from build123d import *

# Parameters (mm, degrees)
STANCHION_PROFILE_SKETCH_R = 17
STANCHION_BODY_DEPTH       = 33
CORNER_NOTCH_SKETCH_W      = 42
CORNER_NOTCH_SKETCH_H      = 58
CORNER_NOTCH_12X12_DEPTH   = 183.247085025
SLOTTED_BOSS_DEPTH         = 8
HINGE_BARREL_SKETCH_R      = 24
HINGE_BARREL_SKETCH_R_2    = 10
HINGE_BARREL_DEPTH         = 27.5
BARREL_START               = -9
BARREL_GUSSET_DEPTH        = 9
BARREL_RECESS_SKETCH_R     = 17
BARREL_RECESS_CUT_DEPTH    = 6


with BuildPart() as part:
    # Stanchion Profile Sketch → Stanchion Body (new, symmetric)
    with BuildSketch(Plane.XY):
        with BuildLine():
            Line((0, 0), (165, 0))
            Line((165, 0), (165, -12))
            Line((165, -12), (149.032106642, -52.311615965))
            ThreePointArc((149.032106642, -52.311615965), (133.013045842, -68.148401729), (110.513423096, -67.061631974))
            Line((110.513423096, -67.061631974), (0, -12))
            Line((0, -12), (0, 0))
        make_face()
        with Locations((123, -42)):
            Circle(STANCHION_PROFILE_SKETCH_R, mode=Mode.SUBTRACT)
    extrude(amount=STANCHION_BODY_DEPTH, both=True)

    # Corner Notch Sketch → Corner Notch 12x12 (cut, through all)
    with BuildSketch(Plane(origin=(165, 0, 0), x_dir=(0, 0, -1), z_dir=(1, 0, 0))):
        with Locations((0, -41)):
            Rectangle(CORNER_NOTCH_SKETCH_W, CORNER_NOTCH_SKETCH_H)
    extrude(amount=-CORNER_NOTCH_12X12_DEPTH, mode=Mode.SUBTRACT)

    # Slotted Boss Sketch → Slotted Boss (add)
    with BuildSketch(Plane(origin=(0, 0, 0), x_dir=(1, 0, 0), z_dir=(0, 1, 0))):
        with BuildLine():
            Line((105, 16), (141, 16))
            ThreePointArc((141, 16), (157, 0), (141, -16))
            Line((141, -16), (105, -16))
            ThreePointArc((105, -16), (89, 0), (105, 16))
        make_face()
        with BuildLine():
            Line((105, 7.5), (141, 7.5))
            ThreePointArc((141, 7.5), (148.5, 0), (141, -7.5))
            Line((141, -7.5), (105, -7.5))
            ThreePointArc((105, -7.5), (97.5, 0), (105, 7.5))
        make_face(mode=Mode.SUBTRACT)
    extrude(amount=SLOTTED_BOSS_DEPTH)



with BuildPart() as body_2:
    # Hinge Barrel Sketch → Hinge Barrel (new, symmetric)
    with BuildSketch(Plane.XY):
        with Locations((50, 45)):
            Circle(HINGE_BARREL_SKETCH_R)
        with Locations((50, 45)):
            Circle(HINGE_BARREL_SKETCH_R_2, mode=Mode.SUBTRACT)
    extrude(amount=HINGE_BARREL_DEPTH, both=True)


with BuildPart() as part_1:
    add(part.part)

    add(body_2.part)  # Barrel Gusset merges body 2
    # Barrel Gusset Sketch → Barrel Gusset (add)
    with BuildSketch(Plane.XY.offset(27.5).offset(BARREL_START)):
        with BuildLine():
            Line((73.619203331, 49.258313517), (82.5, 0))
            Line((82.5, 0), (16.5, 0))
            Line((16.5, 0), (26.468315489, 49.718031802))
            ThreePointArc((26.468315489, 49.718031802), (49.766012583, 21.001140654), (73.619203331, 49.258313517))
        make_face()
    barrel_gusset = extrude(amount=-BARREL_GUSSET_DEPTH)

    # Barrel Gusset Mirror: Barrel Gusset across plane
    add(barrel_gusset.mirror(Plane.XY))

    # Barrel Recess Sketch → Barrel Recess Cut (cut)
    with BuildSketch(Plane.XY.offset(27.5)):
        with Locations((50, 45)):
            Circle(BARREL_RECESS_SKETCH_R)
    barrel_recess_cut = extrude(amount=-BARREL_RECESS_CUT_DEPTH, mode=Mode.SUBTRACT)

    # Barrel Recess Mirror: Barrel Recess Cut across plane
    add(barrel_recess_cut.mirror(Plane.XY), mode=Mode.SUBTRACT)


solid = part_1.part
Verification items for the finished model (mm, model axes). A direction names the side the tool comes from. Give positions to 0.01 mm unless a question says otherwise; leave off trailing zeros. Order: outer loops, then holes, each group sorted by start corner. A loop starts at its lowest first (then second) coordinate and runs counter-clockwise, first axis right, second up. Notation, with made-up numbers: M 47.5,-20.75 L 67.5,-20.75 A8 ccw 67.5,-10.75 Z; hole C 6,65.5 d1. An arc over 180 degrees is marked long. Answer as a JSON object with one key per item and string values. Group by question number.
1) Cross-section at A-A (x = 50). Give the number of separate pieces and of enclosed holes in the cut face, then the cut area to 3 significant figures.
2) Scan lines: line 1 along Z through (x, y) = (24.5, 15); line 2 along Z through (x, y) = (89.5, -41.5); line 3 along Y through (x, z) = (50, 24). Record each from-to range of solid material in increasing order. Write a range as [from, to].
3) Cross-section at C-C (y = -15). Enter the section's corners in (x, z), then the cut area to 3 significant figures.
4) Depth check by flat-ended pin: pin 1 Ø1 at (x, z) = (59.5, -3) entering from -Y; pin 2 Ø5 at (x, z) = (141.5, 21) entering from -Y; pin 3 Ø15 at (x, y) = (38, 33.5) entering from -Z. Enter the tip coordinate at first touch or a pass-through.
5) Cross-section at D-D (x = 123). Enter the section's corners in (y, z), then the cut area to 3 significant figures.
6) Access from +Z, -Z, +X, -X, +Y, -Y to the whole of each face (thin tool, end or side, straight path). Record for faces 4 (the face through (157, 4, 0)), 5 (the face through (102, -35, 21)), 6 (the face through (123, 4, 7.5)), 7 (the face through (57.3, 37.7, 21.5)), 8 (the face through (62.9, 65.24, 0.39)).
7) Cross-section at B-B (z = 0). Enter the section's corners in (x, y).
8) Mould release check, pull along Z, two halves, no side actions. Record for faces 1 (the face through (47.83, 35.24, -0.3)), 2 (the face through (102, -35, -21)), 3 (the face through (84, -27, 33)): released by +Z, released by -Z, zero draft, split by the parting line, or undercut.
Result sheet:
{
 "1": {"separate pieces": "2", "enclosed holes": "1", "area": "3,140 mm2"},
 "2": {"line 1": "z = [-18.5, -9.5], [9.5, 18.5]", "line 2": "z = [-33, -21], [21, 33]", "line 3": "y = [-36.91, 0], [21, 28], [62, 69]"},
 "3": {"outline": "M 6.02,-33 L 163.81,-33 L 163.81,-21 L 6.02,-21 Z; M 6.02,21 L 163.81,21 L 163.81,33 L 6.02,33 Z", "area": "3,790 mm2"},
 "4": {"pin 1": "stops at y = -12", "pin 2": "stops at y = -64.98", "pin 3": "stops at z = -27.5"},
 "5": {"outline": "M -70,-33 L -59,-33 L -59,-21 L -70,-21 Z; M -70,21 L -59,21 L -59,33 L -70,33 Z; M -25,-33 L 0,-33 L 0,-16 L 8,-16 L 8,-7.5 L 0,-7.5 L 0,7.5 L 8,7.5 L 8,16 L 0,16 L 0,33 L -25,33 L -25,21 L -12,21 L -12,-21 L -25,-21 Z", "area": "1,500 mm2"},
 "6": {"face 4": "+X, +Y", "face 5": "+X, -X, -Y", "face 6": "+Y", "face 7": "+Z", "face 8": "none"},
 "7": {"outline": "M 0,-12 L 165,-12 L 165,0 L 157,0 L 157,8 L 148.5,8 L 148.5,0 L 97.5,0 L 97.5,8 L 89,8 L 89,0 L 0,0 Z; C 50,45 d48; hole C 50,45 d20"},
 "8": {"face 1": "zero draft", "face 2": "undercut", "face 3": "released by +Z"}
}
